Build history of the part. All positions in model axes, mm. Give positions to 0.01 mm unless a question says otherwise; leave off trailing zeros. Loops run counter-clockwise (first coordinate to the right, second up) from the corner with the lowest first, then second, coordinate; pieces in that order, holes last. Notation, with made-up numbers: (-39, 0) -> (-24, 0) arc R30 ccw to (-24, 22) -> close; hole circle Ø3 at (-12, 74.25). An arc over 180 degrees is marked (long way). Answer in a Markdown table with one row per item. Add a question column.
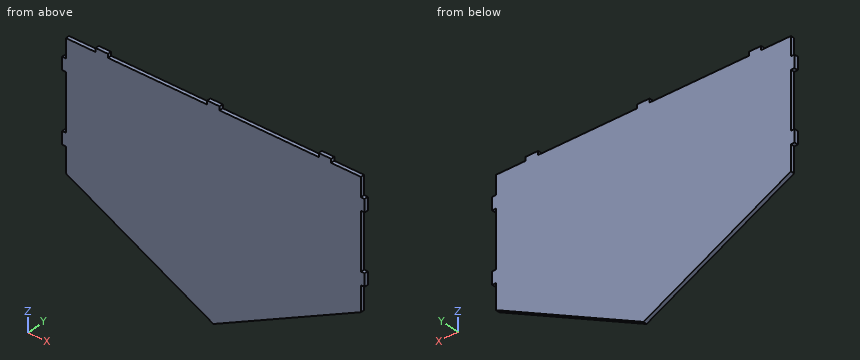
from build123d import *

# Parameters (mm, degrees)
BOSS_EXTRUDE1_DEPTH = 3
SKETCH3_W           = 3
SKETCH3_H           = 10
SKETCH3_W_2         = 10
SKETCH3_H_2         = 3
BOSS_EXTRUDE2_DEPTH = 3


with BuildPart() as part:
    # Sketch1 → Boss-Extrude1 (new body)
    with BuildSketch(Plane(origin=(0, 0, 0), x_dir=(1, 0, 0), z_dir=(0, 1, 0))):
        Polygon((-119, 50), (0, 110), (119, 50), (119, -50), (-119, -50), align=None)
    extrude(amount=BOSS_EXTRUDE1_DEPTH)

    # Sketch3 → Boss-Extrude2 (add)
    with BuildSketch(Plane(origin=(0, 3, 0), x_dir=(1, 0, 0), z_dir=(0, 1, 0))):
        with Locations((120.5, 25)):
            Rectangle(SKETCH3_W, SKETCH3_H)
        with Locations((120.5, -30)):
            Rectangle(SKETCH3_W, SKETCH3_H)
        with Locations((-120.5, -30)):
            Rectangle(SKETCH3_W, SKETCH3_H)
        with Locations((-120.5, 25)):
            Rectangle(SKETCH3_W, SKETCH3_H)
        with Locations((-90, -51.5)):
            Rectangle(SKETCH3_W_2, SKETCH3_H_2)
        with Locations((90, -51.5)):
            Rectangle(SKETCH3_W_2, SKETCH3_H_2)
        with Locations((0, -51.5)):
            Rectangle(SKETCH3_W_2, SKETCH3_H_2)
    extrude(amount=-BOSS_EXTRUDE2_DEPTH)


solid = part.part
(1) Wall check: line 1 along X through (y, z) = (2.4, -12.5); line 2 along Z through (x, y) = (56, 0.2); line 3 along Z through (x, y) = (14, 0.2). Give the ranges that are in metal, low to high. Write a range as from..to.
(2) Saw through at B-B, the plane z = 7.5. List the corners of the cut face in (x, y).
(3) Flat gauge pins, fed straight in: pin 1 Ø0.9 at (x, y) = (-120, 1.5) entering from -Z; pin 2 Ø0.9 at (y, z) = (1.5, 51.5) entering from -X; pin 3 Ø1.5 at (y, z) = (2, -37) entering from +X. Where does each tip first touch, or does it go through?
(4) Saw through at C-C, the plane x = -74.5. List the corners of the cut face in (y, z), then the cut area to 3 significant figures.
Worked answers:
| question | item | result |
|---|---|---|
| 1 | line 1 | -119..119 |
| 1 | line 2 | -81.76..50 |
| 1 | line 3 | -102.94..50 |
| 2 | outline | (-119, 0) -> (119, 0) -> (119, 3) -> (-119, 3) -> close |
| 3 | pin 1 | z = -30 |
| 3 | pin 2 | x = -95 |
| 3 | pin 3 | x = 119 |
| 4 | outline | (0, -72.44) -> (3, -72.44) -> (3, 50) -> (0, 50) -> close |
| 4 | area | 367 mm^2 |
